```python
from build123d import *

# Parameters (mm, degrees)
BOSS_EXTRUDE1_DEPTH = 2113
CUT_EXTRUDE1_REACH  = 2171.532
SKETCH2_R           = 62.5
SKETCH2_W           = 90
SKETCH2_H           = 200
CUT_EXTRUDE2_REACH  = 2156.273
SKETCH3_R           = 25.5


with BuildPart() as part:
    # Sketch1 → Boss-Extrude1 (new body)
    with BuildSketch(Plane.XY):
        with BuildLine():
            Line((0, 0), (300, 0))
            Line((300, 0), (300, 16))
            Line((300, 16), (168, 16))
            ThreePointArc((168, 16), (158.807611845, 19.807611845), (155, 29))
            Line((155, 29), (155, 361))
            ThreePointArc((155, 361), (158.807611845, 370.192388155), (168, 374))
            Line((168, 374), (300, 374))
            Line((300, 374), (300, 390))
            Line((300, 390), (0, 390))
            Line((0, 390), (0, 374))
            Line((0, 374), (132, 374))
            ThreePointArc((132, 374), (141.192388155, 370.192388155), (145, 361))
            Line((145, 361), (145, 29))
            ThreePointArc((145, 29), (141.192388155, 19.807611845), (132, 16))
            Line((132, 16), (0, 16))
            Line((0, 16), (0, 0))
        make_face()
    extrude(amount=BOSS_EXTRUDE1_DEPTH)

    # Sketch2 → Cut-Extrude1 (cut, up to next)
    with BuildSketch(Plane(origin=(0, 390, 0), x_dir=(1, 0, 0), z_dir=(0, 1, 0)), mode=Mode.PRIVATE) as cut_extrude1_sk1:
        with Locations(Location((82, -1986, 0), (0, 0, 270))):
            Circle(SKETCH2_R)
    cut_extrude1_tool1 = extrude(cut_extrude1_sk1.sketch, amount=-CUT_EXTRUDE1_REACH, mode=Mode.PRIVATE) & part.part
    # Sketch2 → Cut-Extrude1 (cut, up to next)
    with BuildSketch(Plane(origin=(0, 390, 0), x_dir=(1, 0, 0), z_dir=(0, 1, 0)), mode=Mode.PRIVATE) as cut_extrude1_sk2:
        with Locations((100, -1723)):
            Rectangle(SKETCH2_W, SKETCH2_H)
    cut_extrude1_tool2 = extrude(cut_extrude1_sk2.sketch, amount=-CUT_EXTRUDE1_REACH, mode=Mode.PRIVATE) & part.part
    add(cut_extrude1_tool1.solids().sort_by_distance((82, 390, 1986))[0], mode=Mode.SUBTRACT)
    add(cut_extrude1_tool2.solids().sort_by_distance((100, 390, 1723))[0], mode=Mode.SUBTRACT)

    # Sketch3 → Cut-Extrude2 (cut, up to next)
    with BuildSketch(Plane.ZY.offset(-145), mode=Mode.PRIVATE) as cut_extrude2_sk1:
        with Locations(Location((1723, 315, 0), (0, 0, 270))):
            Circle(SKETCH3_R)
    cut_extrude2_tool1 = extrude(cut_extrude2_sk1.sketch, amount=-CUT_EXTRUDE2_REACH, mode=Mode.PRIVATE) & part.part
    add(cut_extrude2_tool1.solids().sort_by_distance((145, 315, 1723))[0], mode=Mode.SUBTRACT)


solid = part.part
```
CAD build for the part. Positions are in the model's coordinates, mm. A direction names the side the tool comes from. Round coordinates to 2 decimals unless told otherwise and drop trailing zeros. Loops run counter-clockwise (first coordinate to the right, second up) from the corner with the lowest first, then second, coordinate; pieces in that order, holes last. Notation, with made-up numbers: M 6,2 L 25,2 A29 ccw 25,33 Z; hole C 43,71 d8. An arc over 180 degrees is marked long. Return JSON: item names as keys, results as strings. Group by question number.
(1) Saw through at A-A, the plane z = 1723. List the corners of the cut face in (x, y).
(2) Wall check: probe 1 along Z at (x, y) = (151, 315); probe 2 along X at (y, z) = (378.5, 1986); probe 3 along Y at (x, z) = (288.5, 180). Give the ranges that are in metal, low to high. Write a range as [from, to].
(3) Saw through at C-C, the plane y = 315. List the corners of the cut face in (x, z), and give its area (3 significant figures).
(4) Mould opens along X. For faces 1 (the cylindrical face through (143.968, 380.289, 1977.864)), 2 (the cylindrical face through (149.93, 335.236, 1707.484)), 3 (the flat face through (155, 193, 1042)) say: +X half, -X half, draft (parallel to the pull), parting line (faces both ways), or undercut.
(5) Tool access for faces 4 (the flat face through (65, 374, 807)), 5 (the flat face through (148, 0, 1042)), 6 (the flat face through (235, 16, 1042)): list every direction of +Z, -Z, +X, -X, +Y, -Y with a clear straight run to the whole face (end or side of a thin tool).
(6) Drop flat-ended pins along their axis: P1, Ø6, axis at y = 331, z = 582.5, coming from the +X side; P2, Ø10, axis at y = 252.5, z = 1153, coming from the -X side; P3, Ø10, axis at x = 262.5, z = 1332, coming from the -Y side. Give the stop position or say it passes through.
(7) Saw through at B-B, the plane x = 82. List the corners of the cut face in (y, z), and give its area (3 significant figures).
(8) Saw through at D-D, the plane z = 1986. List the corners of the cut face in (x, y).
Answer list:
{
 "1": {"outline": "M 0,0 L 300,0 L 300,16 L 168,16 A13 cw 155,29 L 155,289.5 L 145,289.5 L 145,29 A13 cw 132,16 L 0,16 Z; M 0,374 L 55,374 L 55,390 L 0,390 Z; M 145,340.5 L 155,340.5 L 155,361 A13 cw 168,374 L 300,374 L 300,390 L 145,390 Z"},
 "2": {"probe 1": "[0, 1697.5], [1748.5, 2113]", "probe 2": "[0, 19.5], [144.5, 300]", "probe 3": "[0, 16], [374, 390]"},
 "3": {"outline": "M 145,0 L 155,0 L 155,1697.5 L 145,1697.5 Z; M 145,1748.5 L 155,1748.5 L 155,2113 L 145,2113 Z", "area": "20,600 mm2"},
 "4": {"face 1": "undercut", "face 2": "draft", "face 3": "+X half"},
 "5": {"face 4": "+Z, -Z, -X", "face 5": "+Z, -Z, +X, -X, -Y", "face 6": "+Z, -Z, +X"},
 "6": {"P1": "x = 155", "P2": "x = 145", "P3": "y = 0"},
 "7": {"outline": "M 0,0 L 16,0 L 16,2113 L 0,2113 Z; M 374,0 L 390,0 L 390,1623 L 374,1623 Z; M 374,1823 L 390,1823 L 390,1923.5 L 374,1923.5 Z; M 374,2048.5 L 390,2048.5 L 390,2113 L 374,2113 Z", "area": "62,400 mm2"},
 "8": {"outline": "M 0,0 L 300,0 L 300,16 L 168,16 A13 cw 155,29 L 155,361 A13 cw 168,374 L 300,374 L 300,390 L 144.5,390 L 144.5,364.57 A13 cw 145,361 L 145,29 A13 cw 132,16 L 0,16 Z; M 0,374 L 19.5,374 L 19.5,390 L 0,390 Z"}
}
